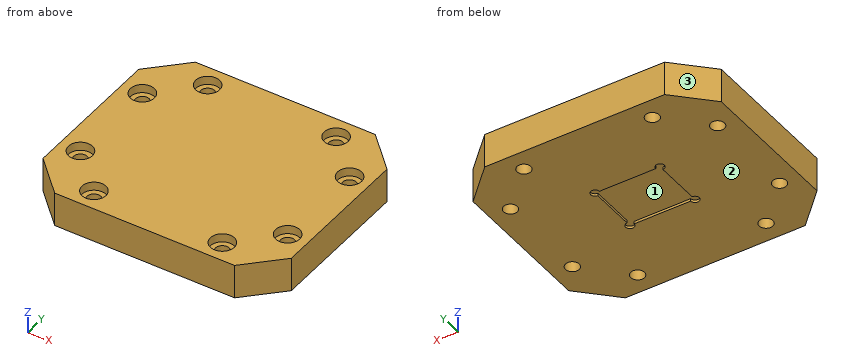
```python
from build123d import *

# Parameters (mm, degrees)
SKETCH_1_W          = 145
SKETCH_1_H          = 125
EXTRUDE_1_DEPTH     = 20
CHAMFER_1_SIZE      = 20
SKETCH_2_R          = 7
CUT_EXTRUDE_1_DEPTH = 5
CUT_EXTRUDE_2_REACH = 98.889
SKETCH_3_R          = 4
SKETCH_4_W          = 38
SKETCH_4_H          = 31
CUT_EXTRUDE_3_DEPTH = 1.5
SKETCH_5_R          = 2.5
CUT_EXTRUDE_4_DEPTH = 1.5


with BuildPart() as part:
    # 草图1 → 凸台-拉伸1 (new body)
    with BuildSketch(Plane.XY):
        Rectangle(SKETCH_1_W, SKETCH_1_H)
    extrude(amount=EXTRUDE_1_DEPTH)

    # 倒角1
    chamfer_1_edges = [part.edges().sort_by_distance(p)[0] for p in [
        (72.5, -62.5, 10),
        (-72.5, -62.5, 10),
        (-72.5, 62.5, 10),
        (72.5, 62.5, 10),
    ]]
    chamfer(chamfer_1_edges, length=CHAMFER_1_SIZE)

    # 草图2 → 切除-拉伸1 (cut)
    with BuildSketch(Plane.XY.offset(20)):
        with Locations((-37.5, 50.5)):
            Circle(SKETCH_2_R)
        with Locations((37.5, 50.5)):
            Circle(SKETCH_2_R)
        with Locations((-60.5, 27.5)):
            Circle(SKETCH_2_R)
        with Locations((-60.5, -27.5)):
            Circle(SKETCH_2_R)
        with Locations((-37.5, -50.5)):
            Circle(SKETCH_2_R)
        with Locations((37.5, -50.5)):
            Circle(SKETCH_2_R)
        with Locations((60.5, 27.5)):
            Circle(SKETCH_2_R)
        with Locations((60.5, -27.5)):
            Circle(SKETCH_2_R)
    extrude(amount=-CUT_EXTRUDE_1_DEPTH, mode=Mode.SUBTRACT)

    # 草图3 → 切除-拉伸2 (cut, up to next)
    with BuildSketch(Plane.XY.offset(15), mode=Mode.PRIVATE) as cut_extrude_2_sk1:
        with Locations((-37.5, 50.5)):
            Circle(SKETCH_3_R)
    cut_extrude_2_tool1 = extrude(cut_extrude_2_sk1.sketch, amount=-CUT_EXTRUDE_2_REACH, mode=Mode.PRIVATE) & part.part
    # 草图3 → 切除-拉伸2 (cut, up to next)
    with BuildSketch(Plane.XY.offset(15), mode=Mode.PRIVATE) as cut_extrude_2_sk2:
        with Locations((-60.5, 27.5)):
            Circle(SKETCH_3_R)
    cut_extrude_2_tool2 = extrude(cut_extrude_2_sk2.sketch, amount=-CUT_EXTRUDE_2_REACH, mode=Mode.PRIVATE) & part.part
    # 草图3 → 切除-拉伸2 (cut, up to next)
    with BuildSketch(Plane.XY.offset(15), mode=Mode.PRIVATE) as cut_extrude_2_sk3:
        with Locations((-60.5, -27.5)):
            Circle(SKETCH_3_R)
    cut_extrude_2_tool3 = extrude(cut_extrude_2_sk3.sketch, amount=-CUT_EXTRUDE_2_REACH, mode=Mode.PRIVATE) & part.part
    # 草图3 → 切除-拉伸2 (cut, up to next)
    with BuildSketch(Plane.XY.offset(15), mode=Mode.PRIVATE) as cut_extrude_2_sk4:
        with Locations((-37.5, -50.5)):
            Circle(SKETCH_3_R)
    cut_extrude_2_tool4 = extrude(cut_extrude_2_sk4.sketch, amount=-CUT_EXTRUDE_2_REACH, mode=Mode.PRIVATE) & part.part
    # 草图3 → 切除-拉伸2 (cut, up to next)
    with BuildSketch(Plane.XY.offset(15), mode=Mode.PRIVATE) as cut_extrude_2_sk5:
        with Locations((37.5, 50.5)):
            Circle(SKETCH_3_R)
    cut_extrude_2_tool5 = extrude(cut_extrude_2_sk5.sketch, amount=-CUT_EXTRUDE_2_REACH, mode=Mode.PRIVATE) & part.part
    # 草图3 → 切除-拉伸2 (cut, up to next)
    with BuildSketch(Plane.XY.offset(15), mode=Mode.PRIVATE) as cut_extrude_2_sk6:
        with Locations((60.5, 27.5)):
            Circle(SKETCH_3_R)
    cut_extrude_2_tool6 = extrude(cut_extrude_2_sk6.sketch, amount=-CUT_EXTRUDE_2_REACH, mode=Mode.PRIVATE) & part.part
    # 草图3 → 切除-拉伸2 (cut, up to next)
    with BuildSketch(Plane.XY.offset(15), mode=Mode.PRIVATE) as cut_extrude_2_sk7:
        with Locations((60.5, -27.5)):
            Circle(SKETCH_3_R)
    cut_extrude_2_tool7 = extrude(cut_extrude_2_sk7.sketch, amount=-CUT_EXTRUDE_2_REACH, mode=Mode.PRIVATE) & part.part
    # 草图3 → 切除-拉伸2 (cut, up to next)
    with BuildSketch(Plane.XY.offset(15), mode=Mode.PRIVATE) as cut_extrude_2_sk8:
        with Locations((37.5, -50.5)):
            Circle(SKETCH_3_R)
    cut_extrude_2_tool8 = extrude(cut_extrude_2_sk8.sketch, amount=-CUT_EXTRUDE_2_REACH, mode=Mode.PRIVATE) & part.part
    add(cut_extrude_2_tool1.solids().sort_by_distance((-37.5, 50.5, 15))[0], mode=Mode.SUBTRACT)
    add(cut_extrude_2_tool2.solids().sort_by_distance((-60.5, 27.5, 15))[0], mode=Mode.SUBTRACT)
    add(cut_extrude_2_tool3.solids().sort_by_distance((-60.5, -27.5, 15))[0], mode=Mode.SUBTRACT)
    add(cut_extrude_2_tool4.solids().sort_by_distance((-37.5, -50.5, 15))[0], mode=Mode.SUBTRACT)
    add(cut_extrude_2_tool5.solids().sort_by_distance((37.5, 50.5, 15))[0], mode=Mode.SUBTRACT)
    add(cut_extrude_2_tool6.solids().sort_by_distance((60.5, 27.5, 15))[0], mode=Mode.SUBTRACT)
    add(cut_extrude_2_tool7.solids().sort_by_distance((60.5, -27.5, 15))[0], mode=Mode.SUBTRACT)
    add(cut_extrude_2_tool8.solids().sort_by_distance((37.5, -50.5, 15))[0], mode=Mode.SUBTRACT)

    # 草图4 → 切除-拉伸3 (cut)
    with BuildSketch(Plane(origin=(0, 0, 0), x_dir=(-1, 0, 0), z_dir=(0, 0, -1))):
        Rectangle(SKETCH_4_W, SKETCH_4_H)
    extrude(amount=-CUT_EXTRUDE_3_DEPTH, mode=Mode.SUBTRACT)

    # 草图5 → 切除-拉伸4 (cut)
    with BuildSketch(Plane(origin=(0, 0, 0), x_dir=(-1, 0, 0), z_dir=(0, 0, -1))):
        with Locations((19, -15.5)):
            Circle(SKETCH_5_R)
        with Locations((-19, -15.5)):
            Circle(SKETCH_5_R)
        with Locations((-19, 15.5)):
            Circle(SKETCH_5_R)
        with Locations((19, 15.5)):
            Circle(SKETCH_5_R)
    extrude(amount=-CUT_EXTRUDE_4_DEPTH, mode=Mode.SUBTRACT)


solid = part.part
```
Geometry check sheet. Reference: the model listing, model coordinates, mm. Face numbers are marked on the shaded views. Coordinates: 2 decimals unless noted, no trailing zeros. Order: outer loops, then holes, each group sorted by start corner. A loop starts at its lowest first (then second) coordinate and runs counter-clockwise, first axis right, second up. Notation, with made-up numbers: (2.5, -17.75) - (51.5, -17.75) arc R18 ccw to (51.5, -13.75) - close; hole circle Ø5 at (11, -11.5). An arc over 180 degrees is marked (long way). Answer in a Markdown table with one row per item. Add a question column.
1. Section check A-A (y = -27.5). Enter the section's corners in (x, z).
2. Section check D-D (x = -7). Enter the section's corners in (y, z), plus the area to 3 significant figures.
3. Section check C-C (z = 6.5). Give the number of separate pieces and of enclosed holes in the cut face, plus the area to 3 significant figures.
4. Draft check along Y on the marked faces 1, 2 and 3. Enter one of: +Y half, -Y half, draft (parallel to the pull), parting line (faces both ways), or undercut.
5. Section check B-B (x = 37.5). Enter the section's corners in (y, z), plus the area to 3 significant figures.
6. Gauge pin test, flat ends, axial feed: pin 1 Ø5 at (x, y) = (-11.5, 9.5) entering from -Z; pin 2 Ø4 at (x, y) = (-39.5, -51.5) entering from +Z. Record the tip position at first contact, or that the pin passes through.
7. Material ranges on L1, parallel to Y at x = 37.5, z = 18.8; L2, parallel to Y at x = -60.5, z = 6.5; L3, parallel to X at y = -49, z = 11, recorded low to high. Write a range as [from, to].
Data:
| question | item | result |
|---|---|---|
| 1 | outline | (-72.5, 0) - (-64.5, 0) - (-64.5, 15) - (-67.5, 15) - (-67.5, 20) - (-72.5, 20) - close; (-56.5, 0) - (56.5, 0) - (56.5, 15) - (53.5, 15) - (53.5, 20) - (-53.5, 20) - (-53.5, 15) - (-56.5, 15) - close; (64.5, 0) - (72.5, 0) - (72.5, 20) - (67.5, 20) - (67.5, 15) - (64.5, 15) - close |
| 2 | outline | (-62.5, 0) - (-15.5, 0) - (-15.5, 1.5) - (15.5, 1.5) - (15.5, 0) - (62.5, 0) - (62.5, 20) - (-62.5, 20) - close |
| 2 | area | 2,450 mm² |
| 3 | separate pieces | 1 |
| 3 | enclosed holes | 8 |
| 3 | area | 16,900 mm² |
| 4 | face 1 | undercut |
| 4 | face 2 | draft |
| 4 | face 3 | +Y half |
| 5 | outline | (-62.5, 0) - (-54.5, 0) - (-54.5, 15) - (-57.5, 15) - (-57.5, 20) - (-62.5, 20) - close; (-46.5, 0) - (46.5, 0) - (46.5, 15) - (43.5, 15) - (43.5, 20) - (-43.5, 20) - (-43.5, 15) - (-46.5, 15) - close; (54.5, 0) - (62.5, 0) - (62.5, 20) - (57.5, 20) - (57.5, 15) - (54.5, 15) - close |
| 5 | area | 2,120 mm² |
| 6 | pin 1 | stops at z = 1.5 |
| 6 | pin 2 | stops at z = 15 |
| 7 | L1 | y = [-62.5, -57.5], [-43.5, 43.5], [57.5, 62.5] |
| 7 | L2 | y = [-54.5, -31.5], [-23.5, 23.5], [31.5, 54.5] |
| 7 | L3 | x = [-66, -41.21], [-33.79, 33.79], [41.21, 66] |
